Work out the finished part from the listing and answer in its coordinate system (mm). A direction names the side the tool comes from. Give positions to 0.01 mm unless a question says otherwise; leave off trailing zeros. Loops run counter-clockwise (first coordinate to the right, second up) from the corner with the lowest first, then second, coordinate; pieces in that order, holes last. Notation, with made-up numbers: M 59,21.5 L 75,21.5 A6 ccw 75,26.5 Z; hole C -14,8 d3. An arc over 180 degrees is marked long. Answer as a JSON object with one key per item and string values. Group by question number.
```python
from build123d import *

# Parameters (mm, degrees)
SKETCH1_R           = 4.75
BOSS_EXTRUDE1_DEPTH = 24.5
SKETCH2_R           = 6
BOSS_EXTRUDE2_DEPTH = 1
CHAMFER1_SIZE       = 0.05
FILLET1_R           = 0.01
CHAMFER2_SIZE       = 0.05
SKETCH4_R           = 5.5
SKETCH4_R_2         = 4.25
CUT_EXTRUDE1_DEPTH  = 1.1


with BuildPart() as part:
    # Sketch1 → Boss-Extrude1 (new body)
    with BuildSketch(Plane(origin=(0, 0, 0), x_dir=(0, 0, -1), z_dir=(1, 0, 0))):
        Circle(SKETCH1_R)
    extrude(amount=BOSS_EXTRUDE1_DEPTH)

    # Sketch2 → Boss-Extrude2 (add)
    with BuildSketch(Plane.ZY):
        Circle(SKETCH2_R)
    extrude(amount=BOSS_EXTRUDE2_DEPTH)

    # Chamfer1
    chamfer1_edges = [part.edges().sort_by_distance(p)[0] for p in [
        (0, 0, -6),
        (-1, 0, -6),
    ]]
    chamfer(chamfer1_edges, length=CHAMFER1_SIZE)

    # Fillet1
    fillet1_edges = [part.edges().sort_by_distance(p)[0] for p in [
        (0, 0, 4.75),
    ]]
    fillet(fillet1_edges, radius=FILLET1_R)

    # Chamfer2
    chamfer2_edges = [part.edges().sort_by_distance(p)[0] for p in [
        (24.5, 0, 4.75),
    ]]
    chamfer(chamfer2_edges, length=CHAMFER2_SIZE)

    # Sketch4 → Cut-Extrude1 (cut)
    with BuildSketch(Plane(origin=(23.5, 0, 0), x_dir=(0, 0, -1), z_dir=(1, 0, 0))):
        Circle(SKETCH4_R)
        Circle(SKETCH4_R_2, mode=Mode.SUBTRACT)
    extrude(amount=-CUT_EXTRUDE1_DEPTH, mode=Mode.SUBTRACT)


solid = part.part
```
Item 1: A tool of negligible diameter and unlimited length cuts with its end or side. For faces 4 (the flat face through (0, 4, -3)), 5 (the flat face through (22.4, -2, 4)), 6 (the flat face through (24.5, 0, 0)), from which of +Z, -Z, +X, -X, +Y, -Y can it reach the whole face along a straight path? Write none if from no direction.
Item 2: Find the intervals of material crossed by probe 1 along X at (y, z) = (0.5, -4.5); probe 2 along Z at (x, y) = (17, -0.25), in increasing order. Write a range as [from, to].
Item 3: A cutting plane is placed at C-C (x = 12.25). Determine the outline of the cut face in (y, z).
Item 4: For a pull along X with two mould halves and no side action, classify faces 1 (the cylindrical face through (11.048, -4.214, -2.192)), 2 (the cylindrical face through (22.958, 3.584, -2.285)), 3 (the flat face through (-1, 0, 0)) as pulls with the +X half, pulls with the -X half, needs draft (parallel to the pull), parting line crosses it, or undercut.
Item 5: Given pin 1 Ø5 at (y, z) = (-5, -2) entering from +X; pin 2 Ø1.5 at (x, z) = (20.5, 0.5) entering from -Y; pin 3 Ø5 at (x, z) = (15, 3.5) entering from +Y; pin 4 Ø3 at (x, y) = (17.5, 3) entering from -Z, each flat-ended and moving along its own axis, determine where each tip first touches the part or whether it passes through.
The answers:
{
 "1": {"face 4": "+X", "face 5": "none", "face 6": "+Z, -Z, +X, +Y, -Y"},
 "2": {"probe 1": "x = [-1, 22.4], [23.5, 24.5]", "probe 2": "z = [-4.74, 4.74]"},
 "3": {"outline": "C 0,0 d9.5"},
 "4": {"face 1": "needs draft", "face 2": "undercut", "face 3": "pulls with the -X half"},
 "5": {"pin 1": "stops at x = 24.5", "pin 2": "stops at y = -4.75", "pin 3": "stops at y = 4.64", "pin 4": "stops at z = -4.51"}
}
